The drawing under review shows one solid part. Ordinate dimensions are in mm from its lowest x, y, z. Coordinates: 2 decimals unless noted, no trailing zeros. Order: outer loops, then holes, each group sorted by start corner. A loop starts at its lowest first (then second) coordinate and runs counter-clockwise, first axis right, second up.
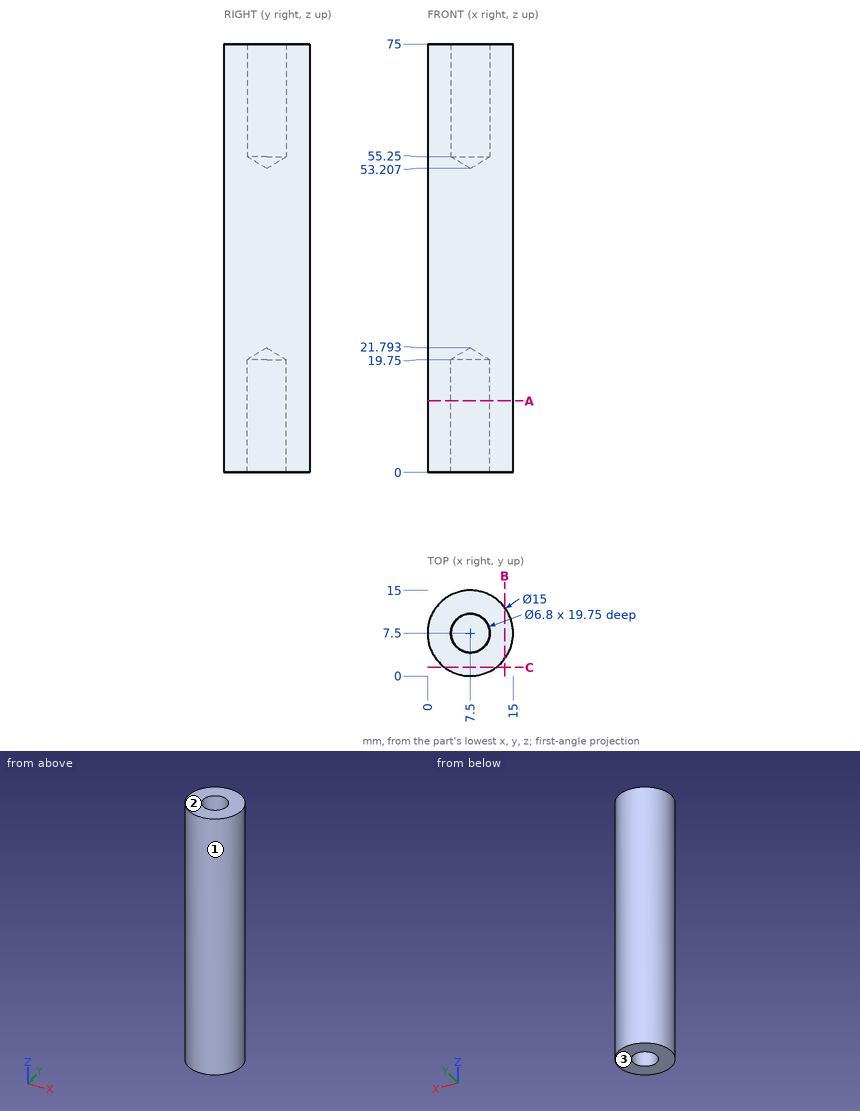
(1) Draft analysis for pull direction Z (two halves, no side actions). For the marked faces 1, 2 and 3, state which applies: released by +Z, released by -Z, zero draft, split by the parting line, or undercut.
A:
face 1: zero draft
face 2: released by +Z
face 3: released by -Z
(2) We need section A-A, the plane z = 12.5. Write out the cut boundary in (x, y), and give its area (3 significant figures).
A:
outline: circle Ø15 at (7.5, 7.5); hole circle Ø6.8 at (7.5, 7.5)
area: 140 mm2
(3) For pin 1 Ø6 at (x, y) = (7.5, 7.5) entering from -Z; pin 2 Ø3 at (x, z) = (3.5, 18) entering from -Y; pin 3 Ø6 at (x, y) = (7.5, 7.5) entering from +Z, all flat-tipped, find the tip position at first contact; note any pin that passes through.
A:
pin 1: stops at z = 19.99
pin 2: stops at y = 0.43
pin 3: stops at z = 55.01
(4) We need section B-B, the plane x = 13.5. Write out the cut boundary in (y, z).
A:
outline: (3, 0) - (12, 0) - (12, 75) - (3, 75) - close
(5) Wall thickness on probe 1 along Y at (x, z) = (7.5, 14); probe 2 along X at (y, z) = (6.75, 13); probe 3 along X at (y, z) = (4.5, 6.5): over which ranges is each line inside the solid? List them lowest first.
A:
probe 1: y = 0 to 4.1, 10.9 to 15
probe 2: x = 0.04 to 4.18, 10.82 to 14.96
probe 3: x = 0.63 to 5.9, 9.1 to 14.37
